Design review of the part shown in the three views and the two pictorial views. Dimensions are in mm from the part's minimum x, y and z. A direction names the side the tool comes from. Coordinates: 2 decimals unless noted, no trailing zeros. Loops run counter-clockwise (first coordinate to the right, second up) from the corner with the lowest first, then second, coordinate; pieces in that order, holes last. Notation, with made-up numbers: M 70,0.5 L 106,0.5 A33 ccw 106,39.5 Z; hole C 24,-37.5 d7. An arc over 180 degrees is marked long. Write item = value, one per line. Start each with the question number.
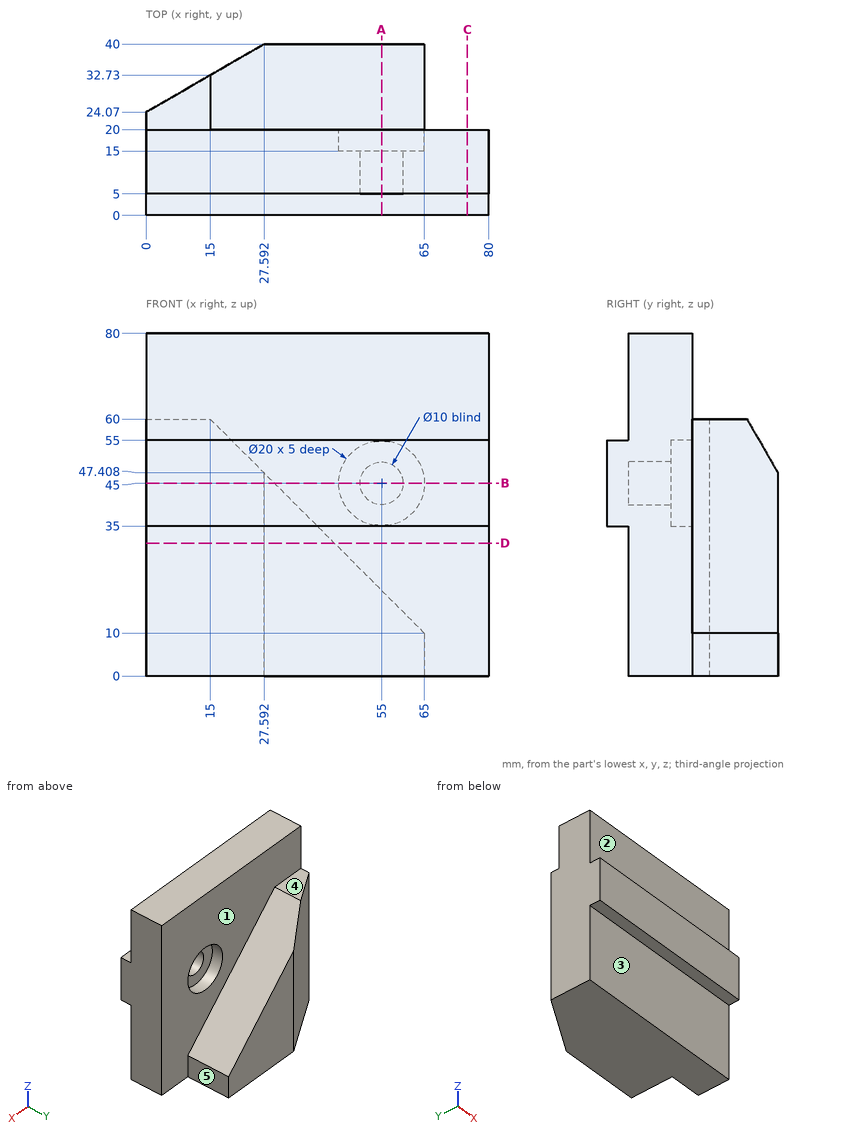
(1) Take a section at C-C (x = 75). State the section outline as (y, z) points.
(2) Take a section at D-D (z = 31). State the section outline as (x, y) points.
(3) Insertion check: pin 1 (4 mm diameter, centred on x = 56.5, y = 1.5, fed in from -Z); pin 2 (1.5 mm diameter, centred on x = 47.5, y = 1.5, fed in from +Z); pin 3 (6.5 mm diameter, centred on x = 6.5, y = 26.5, fed in from +Z). Each pin has a flat end and moves straight along its axis. Give the tip position at first contact, or say it passes through.
(4) Tool access review of the marked faces 1, 2, 3, 4 and 5: name each direction out of +Z, -Z, +X, -X, +Y, -Y from which nothing blocks a thin tool from reaching the whole face with its end or side.
(5) To check wall thickness, follow L1, parallel to X at y = 11.75, z = 45; L2, parallel to Y at x = 40, z = 20; L3, parallel to Y at x = 77, z = 11. State the ranges of each line that lie inside material, in increasing order.
(6) Take a section at A-A (x = 55). State the section outline as (y, z) points.
(7) Take a section at B-B (z = 45). State the section outline as (x, y) points.
Results list:
q1.outline = M 0,35 L 5,35 L 5,0 L 20,0 L 20,80 L 5,80 L 5,55 L 0,55 Z
q2.outline = M 0,5 L 80,5 L 80,20 L 44,20 L 44,40 L 27.59,40 L 0,24.07 Z
q3.pin_1 = 35
q3.pin_2 = 55
q3.pin_3 = 60
q4.face_1 = +Z, +X, +Y
q4.face_2 = +Z, +X, -X, -Y
q4.face_3 = -Z, +X, -X, -Y
q4.face_4 = +Z, +X, -X, +Y
q4.face_5 = +Z, -Z, +X, +Y
q5.L1 = 0 to 50, 60 to 80
q5.L2 = 5 to 40
q5.L3 = 5 to 20
q6.outline = M 0,35 L 5,35 L 5,0 L 40,0 L 40,20 L 20,20 L 20,35 L 15,35 L 15,40 L 5,40 L 5,50 L 15,50 L 15,55 L 20,55 L 20,80 L 5,80 L 5,55 L 0,55 Z
q7.outline = M 0,0 L 80,0 L 80,20 L 65,20 L 65,15 L 60,15 L 60,5 L 50,5 L 50,15 L 45,15 L 45,20 L 30,20 L 30,40 L 27.59,40 L 0,24.07 Z
